```python
from build123d import *


with BuildPart() as part:
    # Sketch 1 → Revolve 1 (revolve)
    with BuildSketch(Plane.XY, mode=Mode.PRIVATE) as revolve_1_sk:
        Polygon((-12.5, 45.5), (-12.5, 19.9), (-22.5, -14.3), (-22.5, -45.5), (-21, -45.5), (-21, -14.514801212), (-11, 19.685198788), (-11, 45.5), align=None)
    revolve(revolve_1_sk.sketch.rotate(Axis((0, 22.245762712, 0), (0, -1, 0)), 270), axis=Axis((0, 22.245762712, 0), (0, -1, 0)))


solid = part.part
```
Source: CAD feature listing. Evaluate the final solid. Frame: model axes, mm. A direction names the side the tool comes from. Round coordinates to 2 decimals unless told otherwise and drop trailing zeros. Loops run counter-clockwise (first coordinate to the right, second up) from the corner with the lowest first, then second, coordinate; pieces in that order, holes last. Notation, with made-up numbers: M 9,80 L 14,80 A20 ccw 14,114 Z; hole C 12.5,60 d11. An arc over 180 degrees is marked long. Use a Markdown table: item, result. Add a question column.
1. Line query: line 1 (X direction, y = -24, z = 0); line 2 (Z direction, x = -1.5, y = -21); line 3 (X direction, y = 27.25, z = 0). Output: solid intervals per line, ascending.
2. Contact query for flat-ended pins moving along their axis: P1, Ø2, axis at y = 14.5, z = 13, coming from the +X side; P2, Ø1, axis at y = 2, z = 2, coming from the -X side; P3, Ø2, axis at x = -13.5, y = 4, coming from the +Z side. Output: stop coordinate, or through.
3. Section query C-C on y = -16. Return the cut outline in (x, z).
4. Reachability of faces 5 (the cylindrical face through (10.74, 32.77, -2.38)), 6 (the cylindrical face through (-3.755, 32.521, 11.923)) from +Z, -Z, +X, -X, +Y, -Y: full face, straight path, thin tool, end or side. Return the list, or none.
5. Section query D-D on y = 11.5. Return the cut outline in (x, z).
6. Section query B-B on z = 0. Return the cut outline in (x, y), then the cut area to 3 significant figures.
7. Section query A-A on x = 0. Return the cut outline in (y, z).
8. Mould query, pull axis X, two halves, no side actions, for faces 1 (the cylindrical face through (-6.31, -29.79, 20.03)), 2 (the cylindrical face through (8.618, -30.118, 20.784)), 3 (the conical face through (9.02, 6.62, -11.76)), 4 (the flat face through (10, 45.5, -5)). Classes: pulls with the +X half, pulls with the -X half, needs draft (parallel to the pull), parting line crosses it, or undercut.
Reported:
| question | item | result |
|---|---|---|
| 1 | line 1 | x = -22.5 to -21, 21 to 22.5 |
| 1 | line 2 | z = -22.45 to -20.95, 20.95 to 22.45 |
| 1 | line 3 | x = -12.5 to -11, 11 to 12.5 |
| 2 | P1 | stops at x = 7.46 |
| 2 | P2 | stops at x = -17.78 |
| 2 | P3 | stops at z = 11.82 |
| 3 | outline | C 0,0 d45; hole C 0,0 d42 |
| 4 | face 5 | +Y, -Y |
| 4 | face 6 | +Y |
| 5 | outline | C 0,0 d29.91; hole C 0,0 d26.79 |
| 6 | outline | M -22.5,-45.5 L -21,-45.5 L -21,-14.51 L -11,19.69 L -11,45.5 L -12.5,45.5 L -12.5,19.9 L -22.5,-14.3 Z; M 11,19.69 L 21,-14.51 L 21,-45.5 L 22.5,-45.5 L 22.5,-14.3 L 12.5,19.9 L 12.5,45.5 L 11,45.5 Z |
| 6 | area | 277 mm² |
| 7 | outline | M -45.5,-22.5 L -14.3,-22.5 L 19.9,-12.5 L 45.5,-12.5 L 45.5,-11 L 19.69,-11 L -14.51,-21 L -45.5,-21 Z; M -45.5,21 L -14.51,21 L 19.69,11 L 45.5,11 L 45.5,12.5 L 19.9,12.5 L -14.3,22.5 L -45.5,22.5 Z |
| 8 | face 1 | undercut |
| 8 | face 2 | parting line crosses it |
| 8 | face 3 | undercut |
| 8 | face 4 | needs draft |
